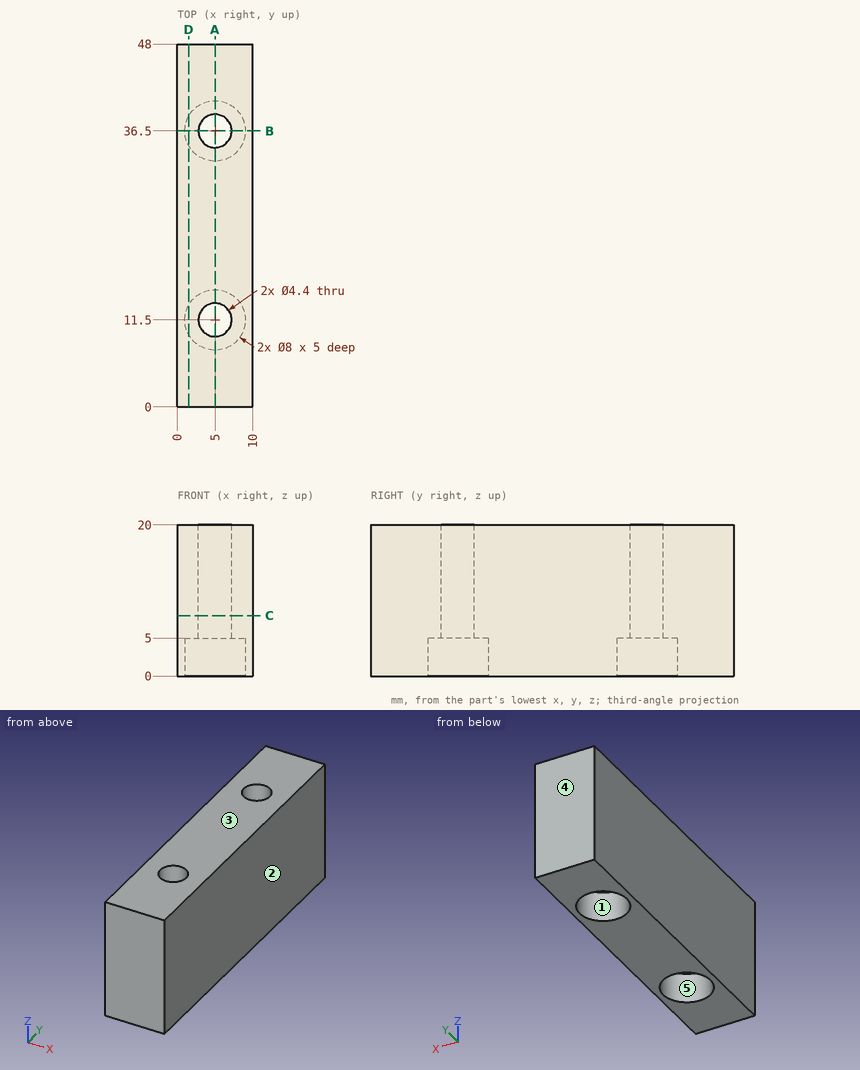
Part print with two shaded views. Sizes in mm from the minimum x, y, z corner. A direction names the side the tool comes from. Give positions to 0.01 mm unless a question says otherwise; leave off trailing zeros. Order: outer loops, then holes, each group sorted by start corner. A loop starts at its lowest first (then second) coordinate and runs counter-clockwise, first axis right, second up. Notation, with made-up numbers: M -5.5,27.25 L -0.5,27.25 A22 ccw -0.5,58.25 Z; hole C -3,-11.5 d5. An arc over 180 degrees is marked long. Write item = value, one per line.
Q1. Cut at C-C, the plane z = 8. List the corners of the cut face in (x, y).
Derived:
outline = M 0,0 L 10,0 L 10,48 L 0,48 Z; hole C 5,11.5 d4.4; hole C 5,36.5 d4.4
Q2. Tool access for the marked faces 1 and 2: list every direction of +Z, -Z, +X, -X, +Y, -Y with a clear straight run to the whole face (end or side of a thin tool).
Derived:
face_1 = -Z
face_2 = +Z, -Z, +X, +Y, -Y
Q3. Cut at B-B, the plane y = 36.5. List the corners of the cut face in (x, z).
Derived:
outline = M 0,0 L 1,0 L 1,5 L 2.8,5 L 2.8,20 L 0,20 Z; M 7.2,5 L 9,5 L 9,0 L 10,0 L 10,20 L 7.2,20 Z
Q4. Drill centre lines: line 1 (Y direction, x = 5, z = 16.75); line 2 (Y direction, x = 5, z = 2.45); line 3 (Z direction, x = 5, y = 8.5). Where is each one in solid material? Low to high. Write a range as [from, to].
Derived:
line_1 = [0, 9.3], [13.7, 34.3], [38.7, 48]
line_2 = [0, 7.5], [15.5, 32.5], [40.5, 48]
line_3 = [5, 20]
Q5. Flat gauge pin, fed straight in: pin 1 (2.5 mm diameter, centred on x = 6, y = 9.5, fed in from -Z). Where does the tip first touch, or does it go through?
Derived:
pin_1 = 5
Q6. Cut at A-A, the plane x = 5. List the corners of the cut face in (y, z), then the cut area to 3 significant figures.
Derived:
outline = M 0,0 L 7.5,0 L 7.5,5 L 9.3,5 L 9.3,20 L 0,20 Z; M 13.7,5 L 15.5,5 L 15.5,0 L 32.5,0 L 32.5,5 L 34.3,5 L 34.3,20 L 13.7,20 Z; M 38.7,5 L 40.5,5 L 40.5,0 L 48,0 L 48,20 L 38.7,20 Z
area = 748 mm2
Q7. Cut at D-D, the plane x = 1.5. List the corners of the cut face in (y, z).
Derived:
outline = M 0,0 L 9.56,0 L 9.56,5 L 13.44,5 L 13.44,0 L 34.56,0 L 34.56,5 L 38.44,5 L 38.44,0 L 48,0 L 48,20 L 0,20 Z
Q8. Two-plate mould, pull along Y, no slides. Class the marked faces 3, 4 and 5: pulls with the +Y half, pulls with the -Y half, needs draft (parallel to the pull), parting line crosses it, or undercut.
Derived:
face_3 = needs draft
face_4 = pulls with the +Y half
face_5 = undercut
